Geometry: final body of the model. Coordinates: model frame, mm. Round coordinates to 2 decimals unless told otherwise and drop trailing zeros. Loops run counter-clockwise (first coordinate to the right, second up) from the corner with the lowest first, then second, coordinate; pieces in that order, holes last. Notation, with made-up numbers: M 7.25,6.25 L 21.25,6.25 A5 ccw 21.25,13.25 Z; hole C 89,-3 d8. An arc over 180 degrees is marked long. Answer as a JSON object with one key per item and string values.
from build123d import *

# Parameters (mm, degrees)
SKETCH_1_W          = 764
SKETCH_1_H          = 860
EXTRUDE_1_DEPTH     = 5
CUT_EXTRUDE_1_REACH = 577.195
SKETCH_2_W          = 280
SKETCH_2_H          = 250


with BuildPart() as part:
    # 草图1 → 凸台-拉伸1 (new body)
    with BuildSketch(Plane.XY):
        Rectangle(SKETCH_1_W, SKETCH_1_H)
    extrude(amount=EXTRUDE_1_DEPTH)

    # 草图2 → 切除-拉伸1 (cut, up to next)
    with BuildSketch(Plane.XY.offset(5), mode=Mode.PRIVATE) as cut_extrude_1_sk1:
        with Locations((-242, -305)):
            Rectangle(SKETCH_2_W, SKETCH_2_H)
    cut_extrude_1_tool1 = extrude(cut_extrude_1_sk1.sketch, amount=-CUT_EXTRUDE_1_REACH, mode=Mode.PRIVATE) & part.part
    add(cut_extrude_1_tool1.solids().sort_by_distance((-242, -305, 5))[0], mode=Mode.SUBTRACT)


solid = part.part
1) Section query C-C (y = -203). Return the cut outline in (x, z).
Results:
{"outline": "M -102,0 L 382,0 L 382,5 L -102,5 Z"}
2) Ray query, line 1 (X direction, y = -283.5, z = 4.2); line 2 (Y direction, x = -141.5, z = 0.45). Return the intervals inside material, ascending.
Results:
{"line 1": "-102 to 382", "line 2": "-180 to 430"}
3) Section query A-A (z = 3.5). Return the cut outline in (x, y).
Results:
{"outline": "M -382,-180 L -102,-180 L -102,-430 L 382,-430 L 382,430 L -382,430 Z"}
4) Pin query (flat end, axial travel): P1, Ø2.5, axis at x = -296.5, z = 3, coming from the -Y side; P2, Ø1.5, axis at y = -340, z = 3, coming from the -X side. Return the tip coordinate at first contact, or that it passes through.
Results:
{"P1": "y = -180", "P2": "x = -102"}
5) Section query B-B (x = -126.5). Return the cut outline in (y, z), and give its area (3 significant figures).
Results:
{"outline": "M -180,0 L 430,0 L 430,5 L -180,5 Z", "area": "3,050 mm2"}
